```python
from build123d import *

# Parameters (mm, degrees)
BOSS_EXTRUDE1_DEPTH = 590
CUT_EXTRUDE1_REACH  = 1573.285


with BuildPart() as part:
    # Sketch1 → Boss-Extrude1 (new body)
    with BuildSketch(Plane.XY):
        Polygon((10, 25), (10, 30), (0, 30), (0, 25), (5, 25), (5, 0), (0, 0), (0, -5), (10, -5), (10, 0), (1446, 0), (1446, -5), (1456, -5), (1456, 0), (1450, 0), (1450, 25), (1456, 25), (1456, 30), (1446, 30), (1446, 25), align=None)
    extrude(amount=BOSS_EXTRUDE1_DEPTH)

    # Sketch2 → Cut-Extrude1 (cut, up to next)
    with BuildSketch(Plane(origin=(0, 25, 0), x_dir=(1, 0, 0), z_dir=(0, 1, 0)), mode=Mode.PRIVATE) as cut_extrude1_sk1:
        Polygon((10, -590), (1446, -590), (1446, -510), (1378.5, -510), (1176, -270), (280, -270), (77.5, -510), (10, -510), align=None)
    cut_extrude1_tool1 = extrude(cut_extrude1_sk1.sketch, amount=-CUT_EXTRUDE1_REACH, mode=Mode.PRIVATE) & part.part
    add(cut_extrude1_tool1.solids().sort_by_distance((728, 25, 443.695445))[0], mode=Mode.SUBTRACT)


solid = part.part
```
Geometry: final body of the model. Coordinates: model frame, mm. A direction names the side the tool comes from. Coordinates: 2 decimals unless noted, no trailing zeros. Write each loop counter-clockwise with the first axis right and the second up, starting at its lowest first coordinate (ties: lowest second). Pieces come first, ordered by that corner, then holes. Notation, with made-up numbers: M 82.5,17 L 137.5,17 A19 cw 137.5,41 Z; hole C 34,-36 d8. An arc over 180 degrees is marked long. Answer as CSV lines item,"result". Start each with the question number.
Q1. Line query: line 1 (X direction, y = -3, z = 224); line 2 (Y direction, x = 893, z = 132.5); line 3 (Z direction, x = 457, y = 10). Output: solid intervals per line, ascending. Write a range as from..to.
Q2. Cut plane D-D on x = 1338. Return the cut outline in (y, z), then the cut area to 4 significant figures.
Q3. Cut plane B-B on y = 11.5. Return the cut outline in (x, z).
Q4. Pin query (flat end, axial travel): P1, Ø20, axis at x = 718.5, y = 13, coming from the +Z side; P2, Ø6, axis at x = 979, z = 225.5, coming from the +Y side; P3, Ø2, axis at y = 22, z = 302.5, coming from the +X side. Return the tip coordinate at first contact, or that it passes through.
Q5. Cut plane A-A on z = 334. Return the cut outline in (x, y), then the cut area to 3 significant figures.
Q6. Reachability of faces 1 (the flat face through (1413, 13, 510)), 2 (the flat face through (1450, 12, 291)), 3 (the flat face through (718, 13, 0)), 4 (the flat face through (10, -1, 359)) from +Z, -Z, +X, -X, +Y, -Y: full face, straight path, thin tool, end or side. Return the list, or none.
Q7. Cut plane C-C on z = 553.5. Return the cut outline in (x, y).
Q8. Mould query, pull axis Y, two halves, no side actions, for faces 5 (the flat face through (180.17, 12.68, 388.32)), 6 (the flat face through (718, 0, 195)), 7 (the flat face through (738, 25, 195)), 8 (the flat face through (5, 13, 291)). Classes: released by +Y, released by -Y, zero draft, split by the parting line, or undercut.
Findings below:
1,line 1,"x = 0..10, 1446..1456"
1,line 2,"y = 0..25"
1,line 3,"z = 0..270"
2,outline,"M 0,0 L 25,0 L 25,462 L 0,462 Z"
2,area,"11,550 mm2"
3,outline,"M 5,0 L 1450,0 L 1450,590 L 1446,590 L 1446,510 L 1378.5,510 L 1176,270 L 280,270 L 77.5,510 L 10,510 L 10,590 L 5,590 Z"
4,P1,"stops at z = 270"
4,P2,"stops at y = 25"
4,P3,"stops at x = 1450"
5,outline,"M 0,-5 L 10,-5 L 10,0 L 226,0 L 226,25 L 10,25 L 10,30 L 0,30 L 0,25 L 5,25 L 5,0 L 0,0 Z; M 1230,0 L 1446,0 L 1446,-5 L 1456,-5 L 1456,0 L 1450,0 L 1450,25 L 1456,25 L 1456,30 L 1446,30 L 1446,25 L 1230,25 Z"
5,area,"11,200 mm2"
6,face 1,"+Z, +Y, -Y"
6,face 2,"+Z, -Z, +X"
6,face 3,"-Z, +X, -X, +Y, -Y"
6,face 4,"+Z"
7,outline,"M 0,-5 L 10,-5 L 10,30 L 0,30 L 0,25 L 5,25 L 5,0 L 0,0 Z; M 1446,-5 L 1456,-5 L 1456,0 L 1450,0 L 1450,25 L 1456,25 L 1456,30 L 1446,30 Z"
8,face 5,"zero draft"
8,face 6,"released by -Y"
8,face 7,"released by +Y"
8,face 8,"undercut"
